Source: CAD feature listing. Evaluate the final solid. Frame: model axes, mm. A direction names the side the tool comes from. Give positions to 0.01 mm unless a question says otherwise; leave off trailing zeros. Loops run counter-clockwise (first coordinate to the right, second up) from the corner with the lowest first, then second, coordinate; pieces in that order, holes last. Notation, with made-up numbers: M -34,11 L 13,11 A19 cw 13,33 Z; hole C -23,54.5 d5. An arc over 180 degrees is marked long. Answer in a Markdown table with one row per item.
```python
from build123d import *

# Parameters (mm, degrees)
BASE_BLOCK_SKETCH_W              = 78
BASE_BLOCK_SKETCH_H              = 12
BASE_BLOCK_DEPTH                 = 50
UPPER_BLOCK_SKETCH_W             = 50
UPPER_BLOCK_SKETCH_H             = 47
UPPER_BLOCK_DEPTH                = 42
STEP_CUT_12MM_DEPTH              = 12
CROSS_HOLE_SKETCH_R              = 8
CROSS_HOLE_DEPTH                 = 50
RECTANGULAR_POCKET_SKETCH_W      = 22
RECTANGULAR_POCKET_SKETCH_H      = 30
RECTANGULAR_THROUGH_POCKET_DEPTH = 80
WEDGE_LUG_DEPTH                  = 50
WEDGE_CUT_A_DEPTH                = 18
WEDGE_CUT_B_DEPTH                = 18


with BuildPart() as part:
    # Base Block Sketch → Base Block (new body)
    with BuildSketch(Plane.XY):
        with Locations((39, -6)):
            Rectangle(BASE_BLOCK_SKETCH_W, BASE_BLOCK_SKETCH_H)
    extrude(amount=BASE_BLOCK_DEPTH)

    # Upper Block Sketch → Upper Block (add)
    with BuildSketch(Plane(origin=(78, 0, 0), x_dir=(0, 0, -1), z_dir=(1, 0, 0))):
        with Locations((-25, 23.5)):
            Rectangle(UPPER_BLOCK_SKETCH_W, UPPER_BLOCK_SKETCH_H)
    extrude(amount=-UPPER_BLOCK_DEPTH)

    # Step Cut Sketch → Step Cut 12mm (cut)
    with BuildSketch(Plane(origin=(0, 0, 0), x_dir=(1, 0, 0), z_dir=(0, 1, 0))):
        with BuildLine():
            Line((25, 0), (0, 0))
            Line((0, 0), (0, -25))
            ThreePointArc((0, -25), (7.32233047, -7.32233047), (25, 0))
        make_face()
        with BuildLine():
            ThreePointArc((25, -50), (7.32233047, -42.67766953), (0, -25))
            Line((0, -25), (0, -50))
            Line((0, -50), (25, -50))
        make_face()
    extrude(amount=-STEP_CUT_12MM_DEPTH, mode=Mode.SUBTRACT)

    # Cross Hole Sketch → Cross Hole (cut)
    with BuildSketch(Plane.XY.offset(50)):
        with Locations((57, 11)):
            Circle(CROSS_HOLE_SKETCH_R)
    extrude(amount=-CROSS_HOLE_DEPTH, mode=Mode.SUBTRACT)

    # Rectangular Pocket Sketch → Rectangular Through Pocket (cut)
    with BuildSketch(Plane(origin=(0, 47, 0), x_dir=(1, 0, 0), z_dir=(0, 1, 0))):
        with Locations((57, -25)):
            Rectangle(RECTANGULAR_POCKET_SKETCH_W, RECTANGULAR_POCKET_SKETCH_H)
    extrude(amount=-RECTANGULAR_THROUGH_POCKET_DEPTH, mode=Mode.SUBTRACT)

    # Wedge Lug Sketch → Wedge Lug (add)
    with BuildSketch(Plane.XY.offset(50)):
        Polygon((36, 47), (0, 0), (36, 0), align=None)
    extrude(amount=-WEDGE_LUG_DEPTH)

    # Wedge Cut A Sketch → Wedge Cut A (cut)
    with BuildSketch(Plane.XY.offset(50)):
        Polygon((36, 47), (36, 0), (0, 0), align=None)
    extrude(amount=-WEDGE_CUT_A_DEPTH, mode=Mode.SUBTRACT)

    # Wedge Cut B Sketch → Wedge Cut B (cut)
    with BuildSketch(Plane(origin=(0, 0, 0), x_dir=(-1, 0, 0), z_dir=(0, 0, -1))):
        Polygon((-36, 47), (-36, 0), (0, 0), align=None)
    extrude(amount=-WEDGE_CUT_B_DEPTH, mode=Mode.SUBTRACT)


solid = part.part
```
1) Section A-A, the plane x = 57. Return loops of the section in (y, z).
Reply:
| item | result |
|---|---|
| outline | M -12,0 L 3,0 L 3,10 L -12,10 Z; M -12,40 L 3,40 L 3,50 L -12,50 Z; M 19,0 L 47,0 L 47,10 L 19,10 Z; M 19,40 L 47,40 L 47,50 L 19,50 Z |
2) Pull-direction query (X, two-part tool) for faces 5 (the cylindrical face through (50.651, 6.132, 45.07)), 6 (the flat face through (36, 24, 9)), 7 (the flat face through (51, 18, 50)); classes: released by +X, released by -X, zero draft, split by the parting line, or undercut.
Reply:
| item | result |
|---|---|
| face 5 | undercut |
| face 6 | released by -X |
| face 7 | zero draft |
3) Pin query (flat end, axial travel): pin 1 Ø9.5 at (x, y) = (57, 11) entering from -Z; pin 2 Ø24 at (x, y) = (57.5, 5.5) entering from +Z; pin 3 Ø14.5 at (y, z) = (20, 7.5) entering from -X; pin 4 Ø9 at (y, z) = (24, 17.5) entering from -X. Return the tip coordinate at first contact, or that it passes through.
Reply:
| item | result |
|---|---|
| pin 1 | passes through |
| pin 2 | stops at z = 50 |
| pin 3 | stops at x = 36 |
| pin 4 | stops at x = 14.96 |
4) Set-up query: faces 1 (the flat face through (26, 13, 18)), 2 (the flat face through (23, 0, 41)), 3 (the flat face through (46, 18, 25)), 4 (the cylindrical face through (50.651, 6.132, 5.07)). Return all of +Z, -Z, +X, -X, +Y, -Y with unobstructed straight access to the full face (end or side cutting, diameter ignored); none if empty.
Reply:
| item | result |
|---|---|
| face 1 | -Z, -X, +Y |
| face 2 | +Z, -X, +Y |
| face 3 | +Y, -Y |
| face 4 | +Z, -Z |
5) Section B-B, the plane y = -4.5. Return loops of the section in (x, z).
Reply:
| item | result |
|---|---|
| outline | M 25,0 L 78,0 L 78,50 L 25,50 A25 ccw Z; hole M 46,10 L 68,10 L 68,40 L 46,40 Z |
6) Section D-D, the plane z = 8.5. Return loops of the section in (x, y).
Reply:
| item | result |
|---|---|
| outline | M 6.22,-12 L 78,-12 L 78,47 L 36,47 L 36,0 L 6.22,0 Z; hole C 57,11 d16 |
7) Material intervals for L1, parallel to Z at x = 51, y = 31; L2, parallel to Y at x = 57, z = 45; L3, parallel to X at y = 27, z = 28, sorted ascending.
Reply:
| item | result |
|---|---|
| L1 | z = 0 to 10, 40 to 50 |
| L2 | y = -12 to 3, 19 to 47 |
| L3 | x = 20.68 to 46, 68 to 78 |
8) Section C-C, the plane z = 31. Return loops of the section in (x, y), then the cut area to 3 significant figures.
Reply:
| item | result |
|---|---|
| outline | M 0,0 L 0.73,0 L 0.73,-12 L 46,-12 L 46,47 L 36,47 Z; M 68,-12 L 78,-12 L 78,47 L 68,47 Z |
| area | 2,450 mm² |
